from build123d import *

# Parameters (mm, degrees)
SKETCH_2_R          = 7.5
CUT_EXTRUDE_1_DEPTH = 2
CUT_EXTRUDE_2_REACH = 95.011
SKETCH_5_R          = 4.5
SKETCH_7_R          = 30.721623485
EXTRUDE_1_DEPTH     = 41
SKETCH_8_R          = 17.5
EXTRUDE_2_DEPTH     = 10
SKETCH_9_R          = 15
EXTRUDE_3_DEPTH     = 45
SKETCH_10_R         = 15
SKETCH_10_R_2       = 13
CUT_EXTRUDE_3_DEPTH = 2


with BuildPart() as part:
    # 草图1 → 旋转1 (revolve)
    with BuildSketch(Plane.XY, mode=Mode.PRIVATE) as revolve_1_sk:
        with BuildLine():
            Line((5, 13.223493336), (5, 0.265127902))
            ThreePointArc((5, 0.265127902), (24.788681465, -14.86973249), (24.233241632, -39.776506664))
            Line((24.233241632, -39.776506664), (55, -39.776506664))
            Line((55, -39.776506664), (55, 13.223493336))
            Line((55, 13.223493336), (5, 13.223493336))
        make_face()
    revolve(revolve_1_sk.sketch.rotate(Axis((0, 13.888286008, 0), (0, -1, 0)), 90), axis=Axis((0, 13.888286008, 0), (0, -1, 0)))

    # 草图2 → 切除-拉伸1 (cut)
    with BuildSketch(Plane.XZ.offset(39.776506664)):
        with Locations(Location((43, 0, 0), (0, 0, 270))):
            Circle(SKETCH_2_R)
        with Locations(Location((30.405591591, -30.405591591, 0), (0, 0, 270))):
            Circle(SKETCH_2_R)
        with Locations(Location((0, -43, 0), (0, 0, 270))):
            Circle(SKETCH_2_R)
        with Locations(Location((-30.405591591, -30.405591591, 0), (0, 0, 270))):
            Circle(SKETCH_2_R)
        with Locations(Location((-43, 0, 0), (0, 0, 270))):
            Circle(SKETCH_2_R)
        with Locations(Location((-30.405591591, 30.405591591, 0), (0, 0, 270))):
            Circle(SKETCH_2_R)
        with Locations(Location((0, 43, 0), (0, 0, 270))):
            Circle(SKETCH_2_R)
        with Locations(Location((30.405591591, 30.405591591, 0), (0, 0, 270))):
            Circle(SKETCH_2_R)
    extrude(amount=-CUT_EXTRUDE_1_DEPTH, mode=Mode.SUBTRACT)

    # 草图5 → 切除-拉伸2 (cut, up to next)
    with BuildSketch(Plane.XZ.offset(37.776506664), mode=Mode.PRIVATE) as cut_extrude_2_sk1:
        with Locations(Location((0, 43, 0), (0, 0, 270))):
            Circle(SKETCH_5_R)
    cut_extrude_2_tool1 = extrude(cut_extrude_2_sk1.sketch, amount=-CUT_EXTRUDE_2_REACH, mode=Mode.PRIVATE) & part.part
    # 草图5 → 切除-拉伸2 (cut, up to next)
    with BuildSketch(Plane.XZ.offset(37.776506664), mode=Mode.PRIVATE) as cut_extrude_2_sk2:
        with Locations(Location((30.405591591, 30.405591591, 0), (0, 0, 270))):
            Circle(SKETCH_5_R)
    cut_extrude_2_tool2 = extrude(cut_extrude_2_sk2.sketch, amount=-CUT_EXTRUDE_2_REACH, mode=Mode.PRIVATE) & part.part
    # 草图5 → 切除-拉伸2 (cut, up to next)
    with BuildSketch(Plane.XZ.offset(37.776506664), mode=Mode.PRIVATE) as cut_extrude_2_sk3:
        with Locations(Location((43, 0, 0), (0, 0, 270))):
            Circle(SKETCH_5_R)
    cut_extrude_2_tool3 = extrude(cut_extrude_2_sk3.sketch, amount=-CUT_EXTRUDE_2_REACH, mode=Mode.PRIVATE) & part.part
    # 草图5 → 切除-拉伸2 (cut, up to next)
    with BuildSketch(Plane.XZ.offset(37.776506664), mode=Mode.PRIVATE) as cut_extrude_2_sk4:
        with Locations(Location((30.405591591, -30.405591591, 0), (0, 0, 270))):
            Circle(SKETCH_5_R)
    cut_extrude_2_tool4 = extrude(cut_extrude_2_sk4.sketch, amount=-CUT_EXTRUDE_2_REACH, mode=Mode.PRIVATE) & part.part
    # 草图5 → 切除-拉伸2 (cut, up to next)
    with BuildSketch(Plane.XZ.offset(37.776506664), mode=Mode.PRIVATE) as cut_extrude_2_sk5:
        with Locations(Location((0, -43, 0), (0, 0, 270))):
            Circle(SKETCH_5_R)
    cut_extrude_2_tool5 = extrude(cut_extrude_2_sk5.sketch, amount=-CUT_EXTRUDE_2_REACH, mode=Mode.PRIVATE) & part.part
    # 草图5 → 切除-拉伸2 (cut, up to next)
    with BuildSketch(Plane.XZ.offset(37.776506664), mode=Mode.PRIVATE) as cut_extrude_2_sk6:
        with Locations(Location((-30.405591591, -30.405591591, 0), (0, 0, 270))):
            Circle(SKETCH_5_R)
    cut_extrude_2_tool6 = extrude(cut_extrude_2_sk6.sketch, amount=-CUT_EXTRUDE_2_REACH, mode=Mode.PRIVATE) & part.part
    # 草图5 → 切除-拉伸2 (cut, up to next)
    with BuildSketch(Plane.XZ.offset(37.776506664), mode=Mode.PRIVATE) as cut_extrude_2_sk7:
        with Locations(Location((-43, 0, 0), (0, 0, 270))):
            Circle(SKETCH_5_R)
    cut_extrude_2_tool7 = extrude(cut_extrude_2_sk7.sketch, amount=-CUT_EXTRUDE_2_REACH, mode=Mode.PRIVATE) & part.part
    # 草图5 → 切除-拉伸2 (cut, up to next)
    with BuildSketch(Plane.XZ.offset(37.776506664), mode=Mode.PRIVATE) as cut_extrude_2_sk8:
        with Locations(Location((-30.405591591, 30.405591591, 0), (0, 0, 270))):
            Circle(SKETCH_5_R)
    cut_extrude_2_tool8 = extrude(cut_extrude_2_sk8.sketch, amount=-CUT_EXTRUDE_2_REACH, mode=Mode.PRIVATE) & part.part
    add(cut_extrude_2_tool1.solids().sort_by_distance((0, -37.776507, 43))[0], mode=Mode.SUBTRACT)
    add(cut_extrude_2_tool2.solids().sort_by_distance((30.405592, -37.776507, 30.405592))[0], mode=Mode.SUBTRACT)
    add(cut_extrude_2_tool3.solids().sort_by_distance((43, -37.776507, 0))[0], mode=Mode.SUBTRACT)
    add(cut_extrude_2_tool4.solids().sort_by_distance((30.405592, -37.776507, -30.405592))[0], mode=Mode.SUBTRACT)
    add(cut_extrude_2_tool5.solids().sort_by_distance((0, -37.776507, -43))[0], mode=Mode.SUBTRACT)
    add(cut_extrude_2_tool6.solids().sort_by_distance((-30.405592, -37.776507, -30.405592))[0], mode=Mode.SUBTRACT)
    add(cut_extrude_2_tool7.solids().sort_by_distance((-43, -37.776507, 0))[0], mode=Mode.SUBTRACT)
    add(cut_extrude_2_tool8.solids().sort_by_distance((-30.405592, -37.776507, 30.405592))[0], mode=Mode.SUBTRACT)

    # 草图7 → 凸台-拉伸1 (add)
    with BuildSketch(Plane.XZ.offset(39.776506664)):
        Circle(SKETCH_7_R)
    extrude(amount=-EXTRUDE_1_DEPTH)

    # 草图8 → 凸台-拉伸2 (add)
    with BuildSketch(Plane.XZ.offset(39.776506664)):
        with Locations(Location((0, 0, 0), (0, 0, 270))):
            Circle(SKETCH_8_R)
    extrude(amount=EXTRUDE_2_DEPTH)

    # 草图9 → 凸台-拉伸3 (add)
    with BuildSketch(Plane.XZ.offset(49.776506664)):
        with Locations(Location((0, 0, 0), (0, 0, 90))):
            Circle(SKETCH_9_R)
    extrude(amount=EXTRUDE_3_DEPTH)

    # 草图10 → 切除-拉伸3 (cut)
    with BuildSketch(Plane.XZ.offset(49.776506664)):
        with Locations(Location((0, 0, 0), (0, 0, 90))):
            Circle(SKETCH_10_R)
        with Locations(Location((0, 0, 0), (0, 0, 270))):
            Circle(SKETCH_10_R_2, mode=Mode.SUBTRACT)
    extrude(amount=CUT_EXTRUDE_3_DEPTH, mode=Mode.SUBTRACT)


solid = part.part
Can you work these out from the model? Positions are in its coordinate system, mm. A direction names the side the tool comes from. Give positions to 0.01 mm unless a question says otherwise; leave off trailing zeros. Loops run counter-clockwise (first coordinate to the right, second up) from the corner with the lowest first, then second, coordinate; pieces in that order, holes last. Notation, with made-up numbers: (-0.75, 64.5) - (4.25, 64.5) arc R30 ccw to (4.25, 99.5) - close; hole circle Ø6 at (34.25, 39.25). An arc over 180 degrees is marked (long way). Answer as a JSON object with one key per item and string values.
Q1. Which directions (+Z, -Z, +X, -X, +Y, -Y) give clear straight access to the entire face, cutting with the end or side of a thin tool? Please do faces 4 (the flat face through (0, 1.223, 0)), 5 (the cylindrical face through (-7.91, -50.763, 10.316)), 6 (the flat face through (-13, -39.777, 13)), 7 (the cylindrical face through (27.7, -12.6, 34)).
Geometry says:
{"face 4": "+Y", "face 5": "none", "face 6": "-Y", "face 7": "+Y, -Y"}
Q2. Will these pins go through, and if not, where does the flat tip stop? P1, Ø1.5, axis at x = -10, z = 24, coming from the -Y side; P2, Ø7, axis at x = 30.41, z = -30.41, coming from the +Y side; P3, Ø11.5, axis at x = -43, z = 0, coming from the -Y side; P4, Ø12, axis at x = -7, y = -12.5, coming from the -Z side.
Geometry says:
{"P1": "y = -39.78", "P2": "through", "P3": "y = -37.78", "P4": "z = -54.99"}
Q3. Imagine slicing it at C-C on y = -17. Give the number of separate pieces and of enclosed holes in the cut face, plus the area to 3 significant figures.
Geometry says:
{"separate pieces": "1", "enclosed holes": "8", "area": "8,990 mm²"}
Q4. Imagine slicing it at A-A on x = -28.5. Write out the boundary of the cut face in (y, z).
Geometry says:
{"outline": "(-39.78, -47.04) - (13.22, -47.04) - (13.22, -34.48) - (-37.78, -34.48) - (-37.78, -37.66) - (-39.78, -37.66) - close; (-39.78, -23.15) - (-37.78, -23.15) - (-37.78, -26.33) - (13.22, -26.33) - (13.22, 26.33) - (-37.78, 26.33) - (-37.78, 23.15) - (-39.78, 23.15) - close; (-39.78, 37.66) - (-37.78, 37.66) - (-37.78, 34.48) - (13.22, 34.48) - (13.22, 47.04) - (-39.78, 47.04) - close"}
Q5. If we mould it in two halves opening along X, with no side actions, what happens to faces 1 (the flat face through (-13.4, -51.777, -0.1)), 2 (the cylindrical face through (-25.944, -12.634, 30.991)), 3 (the cylindrical face through (-0.66, -72.976, -14.985))? For each: pulls with the +X half, pulls with the -X half, needs draft (parallel to the pull), parting line crosses it, or undercut.
Geometry says:
{"face 1": "needs draft", "face 2": "undercut", "face 3": "parting line crosses it"}
Q6. If I drill on L1, parallel to Y at x = 6.5, z = 12; L2, parallel to Z at x = 27, y = -18.5; L3, parallel to Z at x = 34.5, y = -9, over which ranges is the centre line in solid material (lowest first)?
Geometry says:
{"L1": "-94.78 to -51.78, -49.78 to 13.22", "L2": "-47.92 to -33.35, -27.46 to 27.46, 33.35 to 47.92", "L3": "-42.83 to -32.27, -28.54 to 28.54, 32.27 to 42.83"}
Q7. Imagine slicing it at B-B on z = -41.5. Write out the boundary of the cut face in (x, y), plus the area to 3 significant figures.
Geometry says:
{"outline": "(-36.09, -39.78) - (-7.35, -39.78) - (-7.35, -37.78) - (-4.24, -37.78) - (-4.24, 13.22) - (-36.09, 13.22) - close; (4.24, -37.78) - (7.35, -37.78) - (7.35, -39.78) - (36.09, -39.78) - (36.09, 13.22) - (4.24, 13.22) - close", "area": "3,360 mm²"}
Q8. Imagine slicing it at D-D on x = -43. Write out the boundary of the cut face in (y, z).
Geometry says:
{"outline": "(-39.78, -34.29) - (13.22, -34.29) - (13.22, -4.5) - (-37.78, -4.5) - (-37.78, -7.5) - (-39.78, -7.5) - close; (-39.78, 7.5) - (-37.78, 7.5) - (-37.78, 4.5) - (13.22, 4.5) - (13.22, 34.29) - (-39.78, 34.29) - close"}
